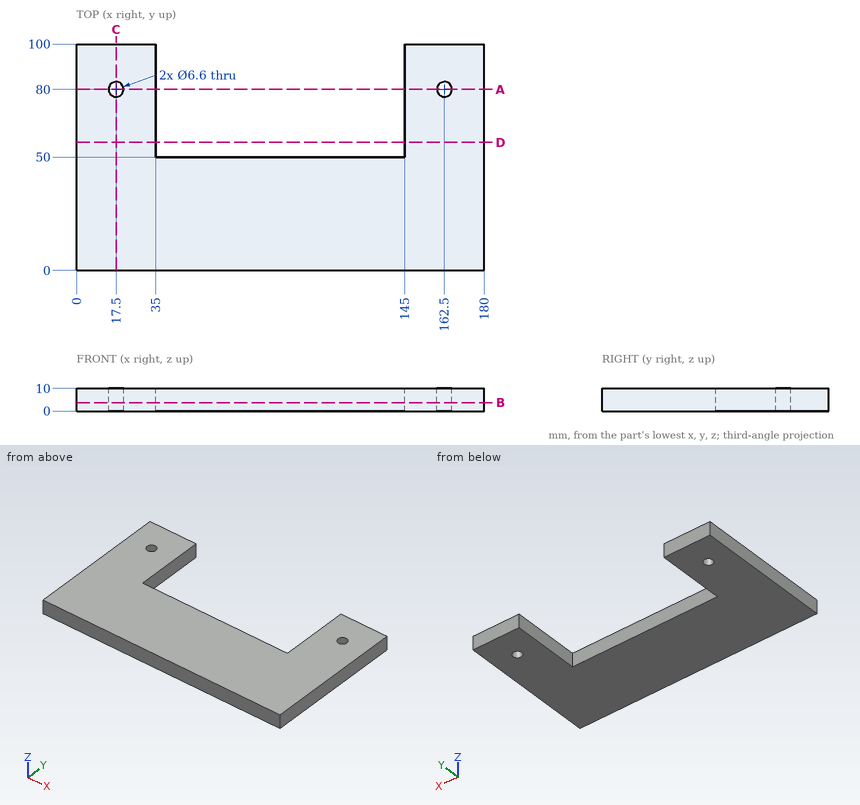
For this review, use the dimensioned drawing (mm, ordinates from the lowest corner) and the shaded views. Coordinates: 2 decimals unless noted, no trailing zeros. Loops run counter-clockwise (first coordinate to the right, second up) from the corner with the lowest first, then second, coordinate; pieces in that order, holes last. Notation, with made-up numbers: (62.5, 78.5) -> (76.5, 78.5) arc R26 cw to (76.5, 93.5) -> close; hole circle Ø10 at (21, 55). An arc over 180 degrees is marked (long way). Use a Markdown table: item, result. Add a question column.
Item 1: We need section B-B, the plane z = 3.75. Write out the cut boundary in (x, y), and give its area (3 significant figures).
Item 2: We need section C-C, the plane x = 17.5. Write out the cut boundary in (y, z), and give its area (3 significant figures).
Item 3: Wall thickness on L1, parallel to X at y = 62.5, z = 6.5; L2, parallel to Y at x = 162.5, z = 7.75; L3, parallel to Y at x = 65.5, z = 8.25: over which ranges is each line inside the solid? List them lowest first. Write a range as from..to.
Item 4: We need section D-D, the plane y = 56.5. Write out the cut boundary in (x, z), and give its area (3 significant figures).
Item 5: Clearance check with flat-ended pins moving along their axes: P1, Ø5.5, axis at x = 162.5, y = 80, coming from the -Z side; P2, Ø1.5, axis at x = 51, z = 6.5, coming from the +Y side. State where each tip first meets the part, or that it passes through.
Item 6: We need section A-A, the plane y = 80. Write out the cut boundary in (x, z).
Numbers:
| question | item | result |
|---|---|---|
| 1 | outline | (0, 0) -> (180, 0) -> (180, 100) -> (145, 100) -> (145, 50) -> (35, 50) -> (35, 100) -> (0, 100) -> close; hole circle Ø6.6 at (17.5, 80); hole circle Ø6.6 at (162.5, 80) |
| 1 | area | 12,400 mm^2 |
| 2 | outline | (0, 0) -> (76.7, 0) -> (76.7, 10) -> (0, 10) -> close; (83.3, 0) -> (100, 0) -> (100, 10) -> (83.3, 10) -> close |
| 2 | area | 934 mm^2 |
| 3 | L1 | x = 0..35, 145..180 |
| 3 | L2 | y = 0..76.7, 83.3..100 |
| 3 | L3 | y = 0..50 |
| 4 | outline | (0, 0) -> (35, 0) -> (35, 10) -> (0, 10) -> close; (145, 0) -> (180, 0) -> (180, 10) -> (145, 10) -> close |
| 4 | area | 700 mm^2 |
| 5 | P1 | passes through |
| 5 | P2 | stops at y = 50 |
| 6 | outline | (0, 0) -> (14.2, 0) -> (14.2, 10) -> (0, 10) -> close; (20.8, 0) -> (35, 0) -> (35, 10) -> (20.8, 10) -> close; (145, 0) -> (159.2, 0) -> (159.2, 10) -> (145, 10) -> close; (165.8, 0) -> (180, 0) -> (180, 10) -> (165.8, 10) -> close |
